from build123d import *

# Parameters (mm, degrees)
HEX_32AF_SKETCH_OUTSIDE_W = 56.456
HEX_32AF_SKETCH_OUTSIDE_H = 56.456
HEX_32AF_CUT_DEPTH        = 25


with BuildPart() as part:
    # Cap Profile Sketch → Cap Body Revolve (revolve)
    with BuildSketch(Plane.XY):
        with BuildLine():
            Line((0, 0), (20, 0))
            Line((20, 0), (20, 20))
            Line((20, 20), (16, 20))
            Line((16, 20), (16, 41))
            ThreePointArc((16, 41), (14.828427125, 43.828427125), (12, 45))
            Line((12, 45), (0, 45))
            Line((0, 45), (0, 0))
        make_face()
    revolve(axis=Axis((0, 0, 0), (0, 1, 0)))

    # Hex 32AF Sketch outside → Hex 32AF Cut (cut)
    with BuildSketch(Plane(origin=(0, 45, 0), x_dir=(1, 0, 0), z_dir=(0, 1, 0))):
        Rectangle(HEX_32AF_SKETCH_OUTSIDE_W, HEX_32AF_SKETCH_OUTSIDE_H)
        Polygon((8, 13.856406461), (-8, 13.856406461), (-16, 0), (-8, -13.856406461), (8, -13.856406461), (16, 0), align=None, mode=Mode.SUBTRACT)
    extrude(amount=-HEX_32AF_CUT_DEPTH, mode=Mode.SUBTRACT)

    # Hex Chamfer 30deg Sketch → Hex Top Chamfer 30deg (revolve, cut)
    with BuildSketch(Plane.XY, mode=Mode.PRIVATE) as hex_top_chamfer_30deg_sk:
        with BuildLine():
            Line((0, 0), (12, 0))
            Line((12, 0), (12, 12))
            Line((12, 12), (9, 13.732050808))
            Line((9, 13.732050808), (9, 39))
            ThreePointArc((9, 39), (8.414213562, 40.414213562), (7, 41))
            Line((7, 41), (0, 41))
            Line((0, 41), (0, 0))
        make_face()
    revolve(hex_top_chamfer_30deg_sk.sketch.rotate(Axis((0, 0, 0), (0, 1, 0)), 90), axis=Axis((0, 0, 0), (0, 1, 0)), mode=Mode.SUBTRACT)


solid = part.part
The listing builds one solid part. Answer for the finished solid, in the listing's coordinates (mm). A direction names the side the tool comes from. Coordinates: 2 decimals unless noted, no trailing zeros. Loops run counter-clockwise (first coordinate to the right, second up) from the corner with the lowest first, then second, coordinate; pieces in that order, holes last. Notation, with made-up numbers: M -2,-22 L 50,-22 A32 ccw 50,16 Z; hole C -24,30.5 d6. An arc over 180 degrees is marked long. Answer in a Markdown table with one row per item.
1) Determine the mould class of faces 1 (the flat face through (0, 41, 0)), 2 (the flat face through (0, 45, 0)), 3 (the flat face through (11.94, 32.44, 7.03)), 4 (the cylindrical face through (-6.083, 26.543, 6.633)) for opening direction Z: released by +Z, released by -Z, zero draft, split by the parting line, or undercut.
Answers below:
| item | result |
|---|---|
| face 1 | undercut |
| face 2 | zero draft |
| face 3 | released by +Z |
| face 4 | undercut |
2) Given pin 1 (4 mm diameter, centred on x = 2.5, z = 1, fed in from -Y); pin 2 (2 mm diameter, centred on x = -11.5, z = -12, fed in from +Y); pin 3 (23.5 mm diameter, centred on x = 0, z = 0, fed in from -Y), each flat-ended and moving along its own axis, determine where each tip first touches the part or whether it passes through.
Answers below:
| item | result |
|---|---|
| pin 1 | y = 41 |
| pin 2 | y = 20 |
| pin 3 | y = 12.14 |
3) Find section C-C (y = 8). Determine the outline of the cut face in (x, z), then the cut area to 3 significant figures.
Answers below:
| item | result |
|---|---|
| outline | C 0,0 d40; hole C 0,0 d24 |
| area | 804 mm^2 |
4) Find section D-D (z = -16.5). Determine the outline of the cut face in (x, y), then the cut area to 3 significant figures.
Answers below:
| item | result |
|---|---|
| outline | M -11.3,0 L 11.3,0 L 11.3,20 L -11.3,20 Z |
| area | 452 mm^2 |
5) Which of the six approach directions +Z, -Z, +X, -X, +Y, -Y give full straight-line access (tool end or side, diameter ignored) to faces 5 (the flat face through (-14, 20, 4)), 6 (the flat face through (0, 32, -13.856)), 7 (the flat face through (-12.056, 32.443, 6.831)), 8 (the flat face through (-11.94, 32.44, -7.03))?
Answers below:
| item | result |
|---|---|
| face 5 | +Y |
| face 6 | -Z, +X, -X, +Y |
| face 7 | +Z, -X, +Y |
| face 8 | -Z, -X, +Y |
6) Find section B-B (x = 0). Determine the outline of the cut face in (y, z).
Answers below:
| item | result |
|---|---|
| outline | M 0,-20 L 20,-20 L 20,-13.86 L 44.54,-13.86 A4 ccw 45,-12 L 45,12 A4 ccw 44.54,13.86 L 20,13.86 L 20,20 L 0,20 L 0,12 L 12,12 L 13.73,9 L 39,9 A2 cw 41,7 L 41,-7 A2 cw 39,-9 L 13.73,-9 L 12,-12 L 0,-12 Z |
7) Find section A-A (y = 21.5). Determine the outline of the cut face in (x, z), then the cut area to 3 significant figures.
Answers below:
| item | result |
|---|---|
| outline | M -16,0 L -8,-13.86 L 8,-13.86 L 16,0 L 8,13.86 L -8,13.86 Z; hole C 0,0 d18 |
| area | 411 mm^2 |
8) Find the intervals of material crossed by probe 1 along X at (y, z) = (33.25, 0); probe 2 along X at (y, z) = (5.25, 0); probe 3 along Y at (x, z) = (0, 7), in increasing order.
Answers below:
| item | result |
|---|---|
| probe 1 | -16 to -9, 9 to 16 |
| probe 2 | -20 to -12, 12 to 20 |
| probe 3 | 41 to 45 |
